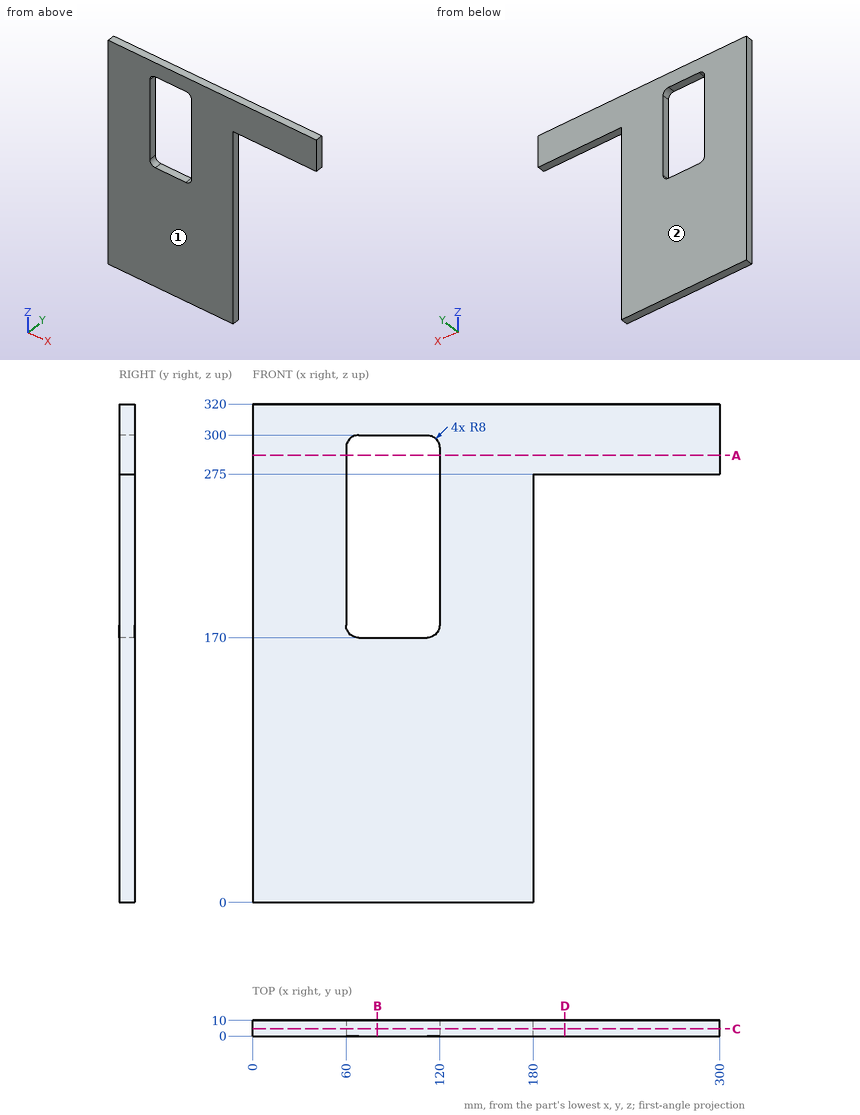
Can you work these out from the drawing? Everything is in mm from the part's minimum corner. Coordinates: 2 decimals unless noted, no trailing zeros. Loops run counter-clockwise (first coordinate to the right, second up) from the corner with the lowest first, then second, coordinate; pieces in that order, holes last.
1) Will these pins go through, and if not, where does the flat tip stop? pin 1 Ø2 at (y, z) = (4.5, 243) entering from -X; pin 2 Ø3 at (y, z) = (4.5, 230) entering from +X.
Reported:
pin 1: stops at x = 0
pin 2: stops at x = 180
2) Imagine slicing it at C-C (y = 4.5). List the corners of the cut face in (x, z) for me.
Reported:
outline: (0, 0) - (180, 0) - (180, 275) - (300, 275) - (300, 320) - (0, 320) - close; hole (60, 178) arc R8 ccw to (68, 170) - (112, 170) arc R8 ccw to (120, 178) - (120, 292) arc R8 ccw to (112, 300) - (68, 300) arc R8 ccw to (60, 292) - close
3) Please list where these lines run through material, in increasing order: line 1 along Z through (x, y) = (76, 1); line 2 along Z through (x, y) = (113, 7.75); line 3 along X through (y, z) = (1, 227.5).
Reported:
line 1: z = 0 to 170, 300 to 320
line 2: z = 0 to 170.06, 299.94 to 320
line 3: x = 0 to 60, 120 to 180
4) Imagine slicing it at D-D (x = 200.5). List the corners of the cut face in (y, z) for me.
Reported:
outline: (0, 275) - (10, 275) - (10, 320) - (0, 320) - close
5) Thinking about a two-plate mould opening in Y: for the marked faces 1 and 2, which applies, released by +Y, released by -Y, zero draft, split by the parting line, or undercut?
Reported:
face 1: released by -Y
face 2: released by +Y
6) Imagine slicing it at B-B (x = 80). List the corners of the cut face in (y, z) for me.
Reported:
outline: (0, 0) - (10, 0) - (10, 170) - (0, 170) - close; (0, 300) - (10, 300) - (10, 320) - (0, 320) - close
7) Imagine slicing it at A-A (z = 287). List the corners of the cut face in (x, y) for me, and give its area (3 significant figures).
Reported:
outline: (0, 0) - (60, 0) - (60, 10) - (0, 10) - close; (120, 0) - (300, 0) - (300, 10) - (120, 10) - close
area: 2,400 mm2
